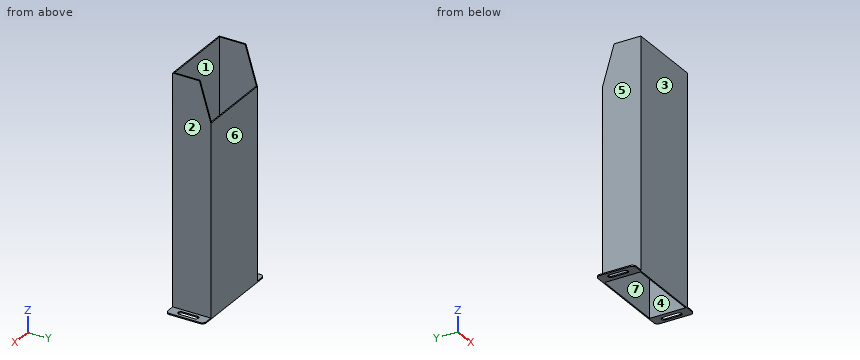
```python
from build123d import *

# Parameters (mm, degrees)
SKETCH_14_W         = 100
SKETCH_14_H         = 50
EXTRUDE_1_DEPTH     = 300
SHELL_1_T           = -1.5
SKETCH_15_W         = 15
SKETCH_15_H         = 50
EXTRUDE_2_DEPTH     = 1.5
CUT_EXTRUDE_1_DEPTH = 323.257660886
FILLET_1_R          = 5
CUT_EXTRUDE_4_DEPTH = 307.51631278
CUT_EXTRUDE_5_REACH = 313.006
SKETCH_21_W         = 97
SKETCH_21_H         = 10


with BuildPart() as part:
    # 草图14 → 凸台-拉伸1 (new body)
    with BuildSketch(Plane.XY):
        Rectangle(SKETCH_14_W, SKETCH_14_H)
    extrude(amount=EXTRUDE_1_DEPTH)

    # 抽壳1
    shell_1_openings = [part.faces().sort_by_distance(p)[0] for p in [
        (0, 0, 300),
        (0, 0, 0),
    ]]
    offset(amount=SHELL_1_T, openings=shell_1_openings, kind=Kind.INTERSECTION)

    # 草图15 → 凸台-拉伸2 (add)
    with BuildSketch(Plane(origin=(0, 0, 0), x_dir=(-1, 0, 0), z_dir=(0, 0, -1))):
        with Locations((-57.5, 0)):
            Rectangle(SKETCH_15_W, SKETCH_15_H)
        with Locations((57.5, 0)):
            Rectangle(SKETCH_15_W, SKETCH_15_H)
    extrude(amount=-EXTRUDE_2_DEPTH)

    # 草图16 → 切除-拉伸1 (cut, through all)
    with BuildSketch(Plane(origin=(50, 0, 0), x_dir=(0, 0, -1), z_dir=(1, 0, 0))):
        Polygon((-300, 10), (-250, 25), (-300, 25), align=None)
    extrude(amount=-CUT_EXTRUDE_1_DEPTH, mode=Mode.SUBTRACT)

    # 圆角1
    fillet_1_edges = [part.edges().sort_by_distance(p)[0] for p in [
        (65, -25, 0.75),
        (65, 25, 0.75),
        (-65, 25, 0.75),
        (-65, -25, 0.75),
    ]]
    fillet(fillet_1_edges, radius=FILLET_1_R)

    # 草图20 → 切除-拉伸4 (cut, through all)
    with BuildSketch(Plane.XY.offset(1.5)):
        with BuildLine():
            Line((-60.75, -10), (-60.75, 10))
            ThreePointArc((-60.75, 10), (-57.5, 13.25), (-54.25, 10))
            Line((-54.25, 10), (-54.25, -10))
            ThreePointArc((-54.25, -10), (-57.5, -13.25), (-60.75, -10))
        make_face()
    cut_extrude_4 = extrude(amount=-CUT_EXTRUDE_4_DEPTH, mode=Mode.SUBTRACT)

    # 镜向1: 切除-拉伸4 across plane
    add(cut_extrude_4.mirror(Plane(origin=(0, 0, 0), x_dir=(0, 0, 1), z_dir=(1, 0, 0))), mode=Mode.SUBTRACT)

    # 草图21 → 切除-拉伸5 (cut, up to next)
    with BuildSketch(Plane(origin=(0, 25, 0), x_dir=(1, 0, 0), z_dir=(0, 1, 0)), mode=Mode.PRIVATE) as cut_extrude_5_sk1:
        with Locations((0, -255)):
            Rectangle(SKETCH_21_W, SKETCH_21_H)
    cut_extrude_5_tool1 = extrude(cut_extrude_5_sk1.sketch, amount=-CUT_EXTRUDE_5_REACH, mode=Mode.PRIVATE) & part.part
    add(cut_extrude_5_tool1.solids().sort_by_distance((0, 25, 255))[0], mode=Mode.SUBTRACT)


solid = part.part
```
Model file for the job. Use its own axes, mm. Face numbers are marked on the shaded views. A direction names the side the tool comes from. Coordinates: 2 decimals unless noted, no trailing zeros. Write each loop counter-clockwise with the first axis right and the second up, starting at its lowest first coordinate (ties: lowest second). Pieces come first, ordered by that corner, then holes. Notation, with made-up numbers: (-9.75, 13.25) - (47.25, 13.25) arc R9 cw to (47.25, 22.25) - close; hole circle Ø10 at (64.5, 5.5). An arc over 180 degrees is marked (long way). Use a Markdown table: item, result. Add a question column.
Item 1: Band-saw the part on C-C, the plane x = 42.5. Write the cut outline in (y, z).
Item 2: Drill centre lines: line 1 along Y through (x, z) = (37, 58.5); line 2 along X through (y, z) = (13, 170); line 3 along Y through (x, z) = (3, 280.5). Where is each one in solid material? Low to high.
Item 3: 3-axis set-ups, long thin cutter, end or side, ignore diameter. For the marked faces 5, 6 and 7: which of +Z, -Z, +X, -X, +Y, -Y reach the whole face in a straight line?
Item 4: Two-plate mould, pull along Y, no slides. Class the marked faces 1, 2, 3 and 4: pulls with the +Y half, pulls with the -Y half, needs draft (parallel to the pull), parting line crosses it, or undercut.
Item 5: Drop flat-ended pins along their axis: pin 1 (7.5 mm diameter, centred on x = 56, y = 8, fed in from +Z); pin 2 (10 mm diameter, centred on y = 13.5, z = 89, fed in from +X); pin 3 (1.2 mm diameter, centred on x = -3.5, y = 24, fed in from +Z); pin 4 (6 mm diameter, centred on x = 3, y = -20, fed in from +Z). Give the stop position or say it passes through.
Item 6: Band-saw the part on B-B, the plane z = 64. Write the cut outline in (x, y), and give its area (3 significant figures).
Item 7: Band-saw the part on A-A, the plane y = 6. Write the cut outline in (x, z), and give its area (4 significant figures).
A:
| question | item | result |
|---|---|---|
| 1 | outline | (-25, 0) - (-23.5, 0) - (-23.5, 300) - (-25, 300) - close; (23.5, 0) - (25, 0) - (25, 250) - (23.5, 250) - close |
| 2 | line 1 | y = -25 to -23.5, 23.5 to 25 |
| 2 | line 2 | x = -50 to -48.5, 48.5 to 50 |
| 2 | line 3 | y = -25 to -23.5 |
| 3 | face 5 | +Z, -X, +Y, -Y |
| 3 | face 6 | +Z, -Z, +X, -X, +Y |
| 3 | face 7 | +Z, -Z |
| 4 | face 1 | undercut |
| 4 | face 2 | needs draft |
| 4 | face 3 | pulls with the -Y half |
| 4 | face 4 | undercut |
| 5 | pin 1 | stops at z = 1.5 |
| 5 | pin 2 | stops at x = 50 |
| 5 | pin 3 | stops at z = 250 |
| 5 | pin 4 | passes through |
| 6 | outline | (-50, -25) - (50, -25) - (50, 25) - (-50, 25) - close; hole (-48.5, -23.5) - (48.5, -23.5) - (48.5, 23.5) - (-48.5, 23.5) - close |
| 6 | area | 441 mm² |
| 7 | outline | (-65, 0) - (-60.75, 0) - (-60.75, 1.5) - (-65, 1.5) - close; (-54.25, 0) - (-48.5, 0) - (-48.5, 300) - (-50, 300) - (-50, 1.5) - (-54.25, 1.5) - close; (48.5, 0) - (54.25, 0) - (54.25, 1.5) - (50, 1.5) - (50, 300) - (48.5, 300) - close; (60.75, 0) - (65, 0) - (65, 1.5) - (60.75, 1.5) - close |
| 7 | area | 925.5 mm² |
